from build123d import *

# Parameters (mm, degrees)
SKETCH1_W             = 53.8
SKETCH1_H             = 10
BOSS_EXTRUDE1_DEPTH   = 29.9
SKETCH2_R             = 1.7
CUT_EXTRUDE1_DEPTH    = 29.9
SKETCH5_W             = 5.4
SKETCH5_H             = 12.8
CUT_EXTRUDE3_DEPTH    = 30
M5_TAPPED_HOLE1_D     = 4.2
M5_TAPPED_HOLE1_DEPTH = 12.4
M5_TAPPED_HOLE1_TIP   = 1.2618073
SKETCH3_W             = 5.8
SKETCH3_H             = 8.2
BOSS_EXTRUDE4_DEPTH   = 11.3
SKETCH7_R             = 0.375
BOSS_EXTRUDE5_DEPTH   = 30
SKETCH8_W             = 10.4
SKETCH8_H             = 34.35
CUT_EXTRUDE4_DEPTH    = 30
SKETCH9_R             = 5
SKETCH9_R_2           = 2
BOSS_EXTRUDE6_DEPTH   = 12.8
FILLET1_R             = 1
FILLET2_R             = 1
CHAMFER2_SIZE         = 5
CHAMFER2_SIZE2        = 1.339745962
SKETCH11_W            = 1
SKETCH11_H            = 1
SKETCH12_R            = 1.75
CUT_EXTRUDE5_DEPTH    = 10
CUT_EXTRUDE6_DEPTH    = 1


with BuildPart() as part:
    # Sketch1 → Boss-Extrude1 (new body)
    with BuildSketch(Plane(origin=(0, 0, 0), x_dir=(0, 0, -1), z_dir=(1, 0, 0))):
        Rectangle(SKETCH1_W, SKETCH1_H)
    extrude(amount=BOSS_EXTRUDE1_DEPTH)

    # Sketch2 → Cut-Extrude1 (cut)
    with BuildSketch(Plane.XZ.offset(5)):
        with Locations(Location((16.3, -19.9, 0), (0, 0, 270))):
            Circle(SKETCH2_R)
        with Locations(Location((16.3, -6.3, 0), (0, 0, 270))):
            Circle(SKETCH2_R)
    extrude(amount=-CUT_EXTRUDE1_DEPTH, mode=Mode.SUBTRACT)

    # Sketch5 → Cut-Extrude3 (cut)
    with BuildSketch(Plane.XZ.offset(5)):
        with Locations((2.7, 20.5)):
            Rectangle(SKETCH5_W, SKETCH5_H)
    extrude(amount=-CUT_EXTRUDE3_DEPTH, mode=Mode.SUBTRACT)

    # M5 Tapped Hole1
    with Locations(Plane(origin=(0, 0, -17.9), x_dir=(0, 0, -1), z_dir=(-1, 0, 0))):
        with Locations((0, 0), (-10.7, 0), (-23, 0)):
            Hole(M5_TAPPED_HOLE1_D / 2, depth=M5_TAPPED_HOLE1_DEPTH)
            with Locations((0, 0, -(M5_TAPPED_HOLE1_DEPTH + M5_TAPPED_HOLE1_TIP / 2))):  # 118° drill point
                Cone(0, M5_TAPPED_HOLE1_D / 2, M5_TAPPED_HOLE1_TIP, mode=Mode.SUBTRACT)

    # Sketch3 → Boss-Extrude4 (add)
    with BuildSketch(Plane.XY.offset(26.9)):
        with Locations((20.15, 0)):
            Rectangle(SKETCH3_W, SKETCH3_H)
    extrude(amount=BOSS_EXTRUDE4_DEPTH)

    # Sketch7 → Boss-Extrude5 (add)
    with BuildSketch(Plane.XY.offset(38.2)):
        with Locations((19.9, 1.25)):
            Circle(SKETCH7_R)
        with Locations((19.9, -1.25)):
            Circle(SKETCH7_R)
    extrude(amount=BOSS_EXTRUDE5_DEPTH)

    # Sketch8 → Cut-Extrude4 (cut)
    with BuildSketch(Plane.XZ.offset(5)):
        with Locations((24.7, -9.725)):
            Rectangle(SKETCH8_W, SKETCH8_H)
    extrude(amount=-CUT_EXTRUDE4_DEPTH, mode=Mode.SUBTRACT)

    # Sketch9 → Boss-Extrude6 (add)
    with BuildSketch(Plane(origin=(19.5, 0, 0), x_dir=(0, 0, -1), z_dir=(1, 0, 0))):
        with Locations(Location((13.1, 0, 0), (0, 0, 270))):
            Circle(SKETCH9_R)
        with Locations((13.1, 0)):
            Circle(SKETCH9_R_2, mode=Mode.SUBTRACT)
    extrude(amount=BOSS_EXTRUDE6_DEPTH)

    # Fillet1
    fillet1_edges = [part.edges().sort_by_distance(p)[0] for p in [
        (32.3, 5, -13.1),
    ]]
    fillet(fillet1_edges, radius=FILLET1_R)

    # Fillet2
    fillet2_edges = [part.edges().sort_by_distance(p)[0] for p in [
        (29.9, 0, 7.45),
    ]]
    fillet(fillet2_edges, radius=FILLET2_R)

    # Chamfer2
    chamfer2_edges = [part.edges().sort_by_distance(p)[0] for p in [
        (29.9, 0, 26.9),
    ]]
    chamfer2_side = [part.faces().sort_by_distance(p)[0] for p in [
        (17.047791734, 0, 26.9),
    ]]
    chamfer(chamfer2_edges, length=CHAMFER2_SIZE, length2=CHAMFER2_SIZE2, reference=chamfer2_side[0])

    # Sketch11 → Cut-Revolve1 (revolve, cut)
    with BuildSketch(Plane(origin=(0, 0, 0), x_dir=(1, 0, 0), z_dir=(0, 1, 0)), mode=Mode.PRIVATE) as cut_revolve1_sk:
        with Locations((29.6, 8.6)):
            Rectangle(SKETCH11_W, SKETCH11_H)
    revolve(cut_revolve1_sk.sketch.rotate(Axis((32.3, 0, -13.1), (-1, 0, 0)), 180), axis=Axis((32.3, 0, -13.1), (-1, 0, 0)), mode=Mode.SUBTRACT)

    # Sketch12 → Cut-Extrude5 (cut)
    with BuildSketch(Plane(origin=(19.5, 0, 0), x_dir=(0, 0, -1), z_dir=(1, 0, 0))):
        with Locations((23.9, 3.1)):
            Circle(SKETCH12_R)
        with Locations((2.3, -3.1)):
            Circle(SKETCH12_R)
    extrude(amount=-CUT_EXTRUDE5_DEPTH, mode=Mode.SUBTRACT)

    # Sketch13 → Cut-Extrude6 (cut)
    with BuildSketch(Plane(origin=(19.5, 0, 0), x_dir=(0, 0, -1), z_dir=(1, 0, 0))):
        with BuildLine():
            Line((4.2, -3.1), (4.2, -5))
            Line((4.2, -5), (0.4, -5))
            Line((0.4, -5), (0.4, -3.1))
            ThreePointArc((0.4, -3.1), (2.3, -1.2), (4.2, -3.1))
        make_face()
        with BuildLine():
            Line((25.852743459, 3.1), (25.852743459, 5))
            Line((25.852743459, 5), (21.947256541, 5))
            Line((21.947256541, 5), (21.947256541, 3.1))
            ThreePointArc((21.947256541, 3.1), (23.9, 1.147256541), (25.852743459, 3.1))
        make_face()
    extrude(amount=-CUT_EXTRUDE6_DEPTH, mode=Mode.SUBTRACT)


solid = part.part
Work out the finished part from the listing and answer in its coordinate system (mm). A direction names the side the tool comes from. Give positions to 0.01 mm unless a question says otherwise; leave off trailing zeros. Loops run counter-clockwise (first coordinate to the right, second up) from the corner with the lowest first, then second, coordinate; pieces in that order, holes last. Notation, with made-up numbers: (60.25, 32.25) -> (77.25, 32.25) arc R17 ccw to (77.25, 44.25) -> close; hole circle Ø10 at (84.25, 6). An arc over 180 degrees is marked (long way). Use a Markdown table: item, result. Add a question column.
1. Section B-B on x = 4 is taken. Determine the outline of the cut face in (y, z).
2. Section C-C on z = 54.5 is taken. Determine the outline of the cut face in (x, y) (3 decimals), and give its area (3 significant figures).
3. Determine the mould class of faces 4 (the flat face through (9.5, -3, -2)), 5 (the flat face through (5.4, 0, 20)), 6 (the flat face through (11, -5, 0)), 7 (the flat face through (30.1, -4, -15)) for opening direction X: released by +X, released by -X, zero draft, split by the parting line, or undercut.
4. Find the intervals of material crossed by probe 1 along Y at (x, z) = (13.5, -23.9); probe 2 along Z at (x, y) = (16.5, -2); probe 3 along Z at (x, y) = (3, 3.75), in increasing order.
5. Section D-D on z = -2.3 is taken. Determine the outline of the cut face in (x, y).
6. For faces 1 (the flat face through (17.25, 0, 32)), 2 (the flat face through (23.05, 0, 32)), 3 (the flat face through (20, -4.1, 32)), determine the directions among +Z, -Z, +X, -X, +Y, -Y from which every point of the face is accessible in a straight line to the end or side of a thin tool.
7. Flat-ended cylindrical pins translate along their axes: pin 1 Ø4 at (y, z) = (2.5, 37.5) entering from -X; pin 2 Ø3 at (y, z) = (3.1, -23.9) entering from +X; pin 3 Ø5.5 at (y, z) = (0, 5.1) entering from +X. Find the tip coordinate at first contact, or state that the pin passes through.
8. Section A-A on x = 16.3 is taken. Determine the outline of the cut face in (y, z), and give its area (3 significant figures).
Results below:
| question | item | result |
|---|---|---|
| 1 | outline | (-5, -26.9) -> (5, -26.9) -> (5, 14.1) -> (-5, 14.1) -> close; hole circle Ø4.2 at (0, -17.9); hole circle Ø4.2 at (0, -7.2); hole circle Ø4.2 at (0, 5.1) |
| 2 | outline | circle Ø0.75 at (19.9, -1.25); circle Ø0.75 at (19.9, 1.25) |
| 2 | area | 0.884 mm^2 |
| 3 | face 4 | released by +X |
| 3 | face 5 | released by -X |
| 3 | face 6 | zero draft |
| 3 | face 7 | undercut |
| 4 | probe 1 | y = -5 to 1.35, 4.85 to 5 |
| 4 | probe 2 | z = -26.9 to -21.59, -18.21 to -7.99, -4.61 to -3.66, -0.94 to 26.9 |
| 4 | probe 3 | z = -26.9 to 14.1 |
| 5 | outline | (0, -5) -> (18.5, -5) -> (18.5, -4.85) -> (9.5, -4.85) -> (9.5, -1.35) -> (18.5, -1.35) -> (18.5, -1.2) -> (19.5, -1.2) -> (19.5, 5) -> (0, 5) -> close |
| 6 | face 1 | +Z, -X, +Y, -Y |
| 6 | face 2 | +Z, +X, +Y, -Y |
| 6 | face 3 | +Z, +X, -X, -Y |
| 7 | pin 1 | stops at x = 17.25 |
| 7 | pin 2 | stops at x = 9.5 |
| 7 | pin 3 | stops at x = 29.7 |
| 8 | outline | (-5, -26.9) -> (5, -26.9) -> (5, -21.6) -> (-5, -21.6) -> close; (-5, -18.2) -> (5, -18.2) -> (5, -8) -> (-5, -8) -> close; (-5, -4.6) -> (5, -4.6) -> (5, 26.9) -> (-5, 26.9) -> close; hole circle Ø3.5 at (-3.1, -2.3); hole circle Ø3.5 at (3.1, -23.9) |
| 8 | area | 451 mm^2 |
